The model under review builds one solid part; all positions refer to its coordinate system, in mm. Coordinates: 2 decimals unless noted, no trailing zeros. Write each loop counter-clockwise with the first axis right and the second up, starting at its lowest first coordinate (ties: lowest second). Pieces come first, ordered by that corner, then holes. Notation, with made-up numbers: (-13, -1.5) - (44, -1.5) arc R9 ccw to (44, 7.5) - close; hole circle Ø2 at (-13, 88). An arc over 180 degrees is marked (long way). Put each result on its own line as item: value. Start each with the question number.
Item 1: Consider section C-C on x = 201. Give the boundary of the cut face in (y, z).
Item 2: Consider section B-B on z = -2. Give the boundary of the cut face in (x, y).
Item 3: To check wall thickness, follow L1, parallel to X at y = 1042.5, z = 0.5; L2, parallel to X at y = 1010, z = 1; L3, parallel to X at y = 779, z = -1. State the ranges of each line that lie inside material, in increasing order. Write a range as [from, to].
Item 4: Consider section A-A on y = 797. Give the boundary of the cut face in (x, z).
Item 5: For pin 1 (1.5 mm diameter, centred on y = 751, z = 1.5, fed in from +X), flat-tipped, find the tip position at first contact; note if it passes through.
```python
from build123d import *

# Parameters (mm, degrees)
SKETCH2_R = 3.25


with BuildPart() as part:
    # Sweep1: sweep along a path in Sketch1
    with BuildLine(Plane.XY) as sweep1_path:
        Line((0, 0), (0, 1133))
        ThreePointArc((0, 1133), (12.30151519, 1162.69848481), (42, 1175))
        Line((42, 1175), (540, 1175))
        ThreePointArc((540, 1175), (569.69848481, 1162.69848481), (582, 1133))
        Line((582, 1133), (582, 964.056768559))
    # Sketch2 → Sweep1 (sweep)
    with BuildSketch(Plane(origin=(0, 0, 0), x_dir=(1, 0, 0), z_dir=(0, 1, 0))):
        Circle(SKETCH2_R)
    sweep(path=sweep1_path.line)


solid = part.part
```
Report:
1. outline: circle Ø6.5 at (1175, 0)
2. outline: (-2.56, 0) - (2.56, 0) - (2.56, 1133) arc R39.44 cw to (42, 1172.44) - (540, 1172.44) arc R39.44 cw to (579.44, 1133) - (579.44, 964.06) - (584.56, 964.06) - (584.56, 1133) arc R44.56 ccw to (540, 1177.56) - (42, 1177.56) arc R44.56 ccw to (-2.56, 1133) - close
3. L1: [-3.21, 3.21], [578.79, 585.21]
3. L2: [-3.09, 3.09], [578.91, 585.09]
3. L3: [-3.09, 3.09]
4. outline: circle Ø6.5 at (0, 0)
5. pin 1: x = 3.16
